from build123d import *

# Parameters (mm, degrees)
SKETCH1_R          = 14.2875
EXTRUDE1_DEPTH     = 25
FILLET1_R          = 6.35
SKETCH2_R          = 8.001
CUT_EXTRUDE1_DEPTH = 92.084332489


with BuildPart() as part:
    # Sketch1 → Extrude1 (new, symmetric)
    with BuildSketch(Plane.XY):
        with BuildLine():
            Line((-25.4, 0), (-25.4, -44.45))
            Line((-25.4, -44.45), (-60.325, -44.45))
            Line((-60.325, -44.45), (-60.325, -63.5))
            Line((-60.325, -63.5), (60.325, -63.5))
            Line((60.325, -63.5), (60.325, -44.45))
            Line((60.325, -44.45), (25.4, -44.45))
            Line((25.4, -44.45), (25.4, 0))
            ThreePointArc((25.4, 0), (0, 25.4), (-25.4, 0))
        make_face()
        Circle(SKETCH1_R, mode=Mode.SUBTRACT)
    extrude(amount=EXTRUDE1_DEPTH, both=True)

    # Fillet1
    fillet1_edges = [part.edges().sort_by_distance(p)[0] for p in [
        (25.4, -44.45, 0),
        (-25.4, -44.45, 0),
    ]]
    fillet(fillet1_edges, radius=FILLET1_R)

    # Sketch2 → Cut-Extrude1 (cut, through all)
    with BuildSketch(Plane(origin=(0, 0, 0), x_dir=(1, 0, 0), z_dir=(0, 1, 0))):
        with Locations(Location((44.45, 0, 0), (0, 0, 270))):
            Circle(SKETCH2_R)
        with Locations(Location((-44.45, 0, 0), (0, 0, 90))):
            Circle(SKETCH2_R)
    extrude(amount=-CUT_EXTRUDE1_DEPTH, mode=Mode.SUBTRACT)


solid = part.part
Could you check a few things on this model? Use its own coordinates, in mm. A direction names the side the tool comes from. Round coordinates to 2 decimals unless told otherwise and drop trailing zeros. Loops run counter-clockwise (first coordinate to the right, second up) from the corner with the lowest first, then second, coordinate; pieces in that order, holes last. Notation, with made-up numbers: (68.25, 9.5) - (80.25, 9.5) arc R20 ccw to (80.25, 34.5) - close; hole circle Ø10 at (24, 9). An arc over 180 degrees is marked (long way). Write item = value, one per line.
1) Imagine slicing it at C-C (y = -48). Please give me the cut outline in (x, z) (3 decimals).
Computed:
outline = (-60.325, -25) - (60.325, -25) - (60.325, 25) - (-60.325, 25) - close; hole circle Ø16.002 at (-44.45, 0); hole circle Ø16.002 at (44.45, 0)
2) I need wall thicknesses on line 1 along X through (y, z) = (-57.25, 0) (3 decimals); line 2 along Y through (x, z) = (0, -2); line 3 along Z through (x, y) = (-44.45, -55.5). Which ranges of each line are inside material? Lowest first, please. Write a range as from..to.
Computed:
line_1 = -60.325..-52.451, -36.449..36.449, 52.451..60.325
line_2 = -63.5..-14.29, 14.29..25.4
line_3 = -25..-8, 8..25
3) On a 3-axis mill with a long thin cutter (end or side, diameter ignored), from which of +Z, -Z, +X, -X, +Y, -Y can I reach the whole of each face in a straight line? I mean faces 4 (the flat face through (25.4, -19, 0)), 5 (the flat face through (-25.4, -19, 0)), 6 (the flat face through (-1, -38, -25)). Say none if no direction works.
Computed:
face_4 = +Z, -Z, +X, +Y
face_5 = +Z, -Z, -X, +Y
face_6 = -Z, +X, -X, +Y, -Y
4) If we mould it in two halves opening along Y, with no side actions, what happens to faces 1 (the cylindrical face through (36.64, -53.84, -1.73)), 2 (the cylindrical face through (-14.274, 0.628, -0.35)), 3 (the cylindrical face through (27.21, -42.54, -0.35))? For each: pulls with the +Y half, pulls with the -Y half, needs draft (parallel to the pull), parting line crosses it, or undercut.
Computed:
face_1 = needs draft
face_2 = undercut
face_3 = pulls with the +Y half
5) Imagine slicing it at B-B (x = 44.45). Please give me the cut outline in (y, z).
Computed:
outline = (-63.5, -25) - (-44.45, -25) - (-44.45, -8) - (-63.5, -8) - close; (-63.5, 8) - (-44.45, 8) - (-44.45, 25) - (-63.5, 25) - close
6) Imagine slicing it at A-A (z = 0). Give the number of separate pieces and of enclosed holes in the cut face, and give its area (3 significant figures).
Computed:
separate_pieces = 3
enclosed_holes = 1
area = 4,340 mm2
7) Imagine slicing it at D-D (y = -3). Please give me the cut outline in (x, z).
Computed:
outline = (-25.4, -25) - (-13.97, -25) - (-13.97, 25) - (-25.4, 25) - close; (13.97, -25) - (25.4, -25) - (25.4, 25) - (13.97, 25) - close
8) I'm going to push flat-ended pins straight in: P1, Ø21, axis at x = -44.45, z = 0, coming from the +Y side; P2, Ø8, axis at y = -37, z = 5.5, coming from the +X side; P3, Ø19, axis at y = -28, z = -1.5, coming from the -X side; P4, Ø1.5, axis at x = 45.5, z = -7, coming from the -Y side. Where does each tip first touch, or does it pass through?
Computed:
P1 = -44.45
P2 = 26.1
P3 = -25.4
P4 = through
